from build123d import *

# Parameters (mm, degrees)
SKETCH1_R                               = 41
BOSS_EXTRUDE1_DEPTH                     = 16.5
SKETCH2_R                               = 36.975
BOSS_EXTRUDE2_DEPTH                     = 1.5
SKETCH4_W                               = 50
SKETCH4_H                               = 6.84002239
CUT_EXTRUDE1_DEPTH                      = 61.712436947
SKETCH5_R                               = 31
CUT_EXTRUDE3_DEPTH                      = 8
SKETCH6_R                               = 29
CUT_EXTRUDE4_DEPTH                      = 8
CUT_EXTRUDE5_DEPTH                      = 57.108382841
CUT_EXTRUDE5_DEPTH_BACK                 = 57.108382841
CBORE_FOR_M3_HEX_HEAD_BOLT3_D           = 3.5
CBORE_FOR_M3_HEX_HEAD_BOLT3_CBORE_D     = 6
CBORE_FOR_M3_HEX_HEAD_BOLT3_CBORE_DEPTH = 4
M3_TAPPED_HOLE1_D                       = 2.5
CIRPATTERN1_COUNT                       = 3


with BuildPart() as part:
    # Sketch1 → Boss-Extrude1 (new body)
    with BuildSketch(Plane.XY):
        Circle(SKETCH1_R)
    extrude(amount=BOSS_EXTRUDE1_DEPTH)

    # Sketch2 → Boss-Extrude2 (add)
    with BuildSketch(Plane(origin=(0, 0, 0), x_dir=(-1, 0, 0), z_dir=(0, 0, -1))):
        Circle(SKETCH2_R)
    extrude(amount=BOSS_EXTRUDE2_DEPTH)

    # Sketch4 → Cut-Extrude1 (cut, through all)
    with BuildSketch(Plane(origin=(0, 0, -1.5), x_dir=(-1, 0, 0), z_dir=(0, 0, -1))):
        with Locations((0, 40.395011195)):
            Rectangle(SKETCH4_W, SKETCH4_H)
        with Locations((0, -40.395011195)):
            Rectangle(SKETCH4_W, SKETCH4_H)
    extrude(amount=-CUT_EXTRUDE1_DEPTH, mode=Mode.SUBTRACT)

    # Sketch5 → Cut-Extrude3 (cut)
    with BuildSketch(Plane(origin=(0, 0, -1.5), x_dir=(-1, 0, 0), z_dir=(0, 0, -1))):
        Circle(SKETCH5_R)
    extrude(amount=-CUT_EXTRUDE3_DEPTH, mode=Mode.SUBTRACT)

    # Sketch6 → Cut-Extrude4 (cut)
    with BuildSketch(Plane.XY.offset(16.5)):
        Circle(SKETCH6_R)
    extrude(amount=-CUT_EXTRUDE4_DEPTH, mode=Mode.SUBTRACT)

    # Sketch7 → Cut-Extrude5 (cut, two sides: drawn at the far end of the back side and taken through both)
    with BuildSketch(Plane.XY.offset(8.5).offset(-CUT_EXTRUDE5_DEPTH_BACK)):
        with BuildLine():
            Line((0, 18), (36.837480913, 18))
            ThreePointArc((36.837480913, 18), (41, 0), (36.837480913, -18))
            Line((36.837480913, -18), (0, -18))
            ThreePointArc((0, -18), (-18, 0), (0, 18))
        make_face()
    extrude(amount=CUT_EXTRUDE5_DEPTH + CUT_EXTRUDE5_DEPTH_BACK, mode=Mode.SUBTRACT)

    # CBORE for M3 Hex Head Bolt3 (through all)
    with Locations(Plane(origin=(0, 34, 16.5), x_dir=(1, 0, 0), z_dir=(0, 0, 1))):
        with Locations((0, 0), (0, -68)):
            CounterBoreHole(CBORE_FOR_M3_HEX_HEAD_BOLT3_D / 2, CBORE_FOR_M3_HEX_HEAD_BOLT3_CBORE_D / 2, CBORE_FOR_M3_HEX_HEAD_BOLT3_CBORE_DEPTH)

    # M3 Tapped Hole1 (through all)
    with Locations(Plane(origin=(-35, 0, 16.5), x_dir=(1, 0, 0), z_dir=(0, 0, 1))):
        with Locations((0, 0)):
            m3_tapped_hole1 = Hole(M3_TAPPED_HOLE1_D / 2)

    # CirPattern1: M3 Tapped Hole1 ×3 about axis
    cirpattern1_axis = Axis((0, 0, 0), (0, 0, 1))
    for i in range(1, CIRPATTERN1_COUNT):
        add(m3_tapped_hole1.rotate(cirpattern1_axis, i * 360 / CIRPATTERN1_COUNT), mode=Mode.SUBTRACT)


solid = part.part
Work out the finished part from the listing and answer in its coordinate system (mm). A direction names the side the tool comes from. Coordinates: 2 decimals unless noted, no trailing zeros. Order: outer loops, then holes, each group sorted by start corner. A loop starts at its lowest first (then second) coordinate and runs counter-clockwise, first axis right, second up. Notation, with made-up numbers: (30.25, 60.25) - (67.25, 60.25) arc R16 ccw to (67.25, 82.25) - close; hole circle Ø6 at (57.25, 11.25). An arc over 180 degrees is marked (long way). Put each result on its own line as item: value. Start each with the question number.
1) Find the intervals of material crossed by line 1 (Y direction, x = 0, z = 10.75) (3 decimals); line 2 (Y direction, x = 0, z = 3.75) (3 decimals); line 3 (Y direction, x = -10, z = 10.25) (3 decimals), in increasing order. Write a range as from..to.
2) Flat-ended cylindrical pins translate along their axes: pin 1 (3 mm diameter, centred on x = 0, y = -34, fed in from +Z); pin 2 (6 mm diameter, centred on y = 19, z = 8.5, fed in from +X); pin 3 (1.5 mm diameter, centred on x = -3, y = -22, fed in from -Z); pin 4 (3 mm diameter, centred on y = 3, z = 8.5, fed in from -X). Find the tip coordinate at first contact, or state that the pin passes through.
3) For a pull along X with two mould halves and no side action, classify faces 1 (the flat face through (0, 36.975, 8)), 2 (the cylindrical face through (28.74, -29.24, 8.13)), 3 (the cylindrical face through (-28.983, 1.003, 12.556)) as released by +X, released by -X, zero draft, split by the parting line, or undercut.
4) Find section D-D (x = -23.5). Give the vertices of the cut face in (y, z).
5) Find section B-B (y = 30). Give the vertices of the cut face in (x, z), plus the area to 3 significant figures.
6) Find section C-C (z = 9.5). Give the vertices of the cut face in (x, y) (3 decimals), plus the area to 3 significant figures.
7) For faces 4 (the flat face through (-37.3, 0.2, 0)), 5 (the flat face through (26, 18, 7)), 6 (the cylindrical face through (-30.98, -1.09, 2.44)), 7 (the flat face through (1.3, 35.4, 12.5)), determine the directions among +Z, -Z, +X, -X, +Y, -Y from which every point of the face is accessible in a straight line to the end or side of a thin tool.
8) Find section A-A (x = 5). Give the vertices of the cut face in (y, z) (3 decimals).
Results list:
1. line 1: y = -36.975..-35.75, -32.25..-29, 29..32.25, 35.75..36.975
1. line 2: y = -36.975..-35.75, -32.25..-31, 31..32.25, 35.75..36.975
1. line 3: y = -36.975..-27.221, 27.221..36.975
2. pin 1: passes through
2. pin 2: stops at x = 36.84
2. pin 3: stops at z = 6.5
2. pin 4: stops at x = -40.97
3. face 1: zero draft
3. face 2: released by +X
3. face 3: undercut
4. outline: (-33.6, 0) - (-28.55, 0) - (-28.55, -1.5) - (-20.22, -1.5) - (-20.22, 6.5) - (20.22, 6.5) - (20.22, -1.5) - (28.55, -1.5) - (28.55, 0) - (33.6, 0) - (33.6, 16.5) - (16.99, 16.5) - (16.99, 8.5) - (-16.99, 8.5) - (-16.99, 16.5) - (-33.6, 16.5) - close
5. outline: (-27.95, 0) - (-21.61, 0) - (-21.61, -1.5) - (-7.81, -1.5) - (-7.81, 6.5) - (7.81, 6.5) - (7.81, -1.5) - (16.29, -1.5) - (16.29, 16.5) - (-27.95, 16.5) - close; (18.71, -1.5) - (21.61, -1.5) - (21.61, 0) - (27.95, 0) - (27.95, 16.5) - (18.71, 16.5) - close
5. area: 819 mm^2
6. outline: (-17.716, -36.975) - (17.716, -36.975) arc R41 ccw to (36.837, -18) - (22.738, -18) arc R29 cw (long way) to (22.738, 18) - (36.837, 18) arc R41 ccw to (17.716, 36.975) - (-17.716, 36.975) arc R41 ccw to start; hole circle Ø2.5 at (-35, 0); hole circle Ø3.5 at (0, -34); hole circle Ø3.5 at (0, 34); hole circle Ø2.5 at (17.5, -30.311); hole circle Ø2.5 at (17.5, 30.311)
6. area: 1,960 mm^2
7. face 4: -Z, -X
7. face 5: +Z, -Z, +X
7. face 6: -Z
7. face 7: +Z
8. outline: (-36.975, 0) - (-36.635, 0) - (-36.635, -1.5) - (-30.594, -1.5) - (-30.594, 6.5) - (-18, 6.5) - (-18, 8.5) - (-28.566, 8.5) - (-28.566, 16.5) - (-36.975, 16.5) - close; (18, 6.5) - (30.594, 6.5) - (30.594, -1.5) - (36.635, -1.5) - (36.635, 0) - (36.975, 0) - (36.975, 16.5) - (28.566, 16.5) - (28.566, 8.5) - (18, 8.5) - close
